Part model, mm, in its own coordinate system. A direction names the side the tool comes from. Round coordinates to 2 decimals unless told otherwise and drop trailing zeros. Loops run counter-clockwise (first coordinate to the right, second up) from the corner with the lowest first, then second, coordinate; pieces in that order, holes last.
from build123d import *

# Parameters (mm, degrees)
SKETCH_1_W                     = 248
SKETCH_1_H                     = 60
EXTRUDE_1_DEPTH                = 6
HOLE_WIZARD_M5_1_D             = 4.2
HOLE_WIZARD_M5_1_DEPTH         = 12.4
HOLE_WIZARD_M5_1_TIP           = 1.2618073
CHAMFER_1_SIZE                 = 2
HOLE_WIZARD_M5_1_2_D           = 5.5
HOLE_WIZARD_M5_1_2_DEPTH       = 12.4
HOLE_WIZARD_M5_1_2_CBORE_D     = 10
HOLE_WIZARD_M5_1_2_CBORE_DEPTH = 5.7
HOLE_WIZARD_M5_1_2_TIP         = 1.652366702


with BuildPart() as part:
    # 草图1 → 凸台-拉伸1 (new, symmetric)
    with BuildSketch(Plane.XY):
        Rectangle(SKETCH_1_W, SKETCH_1_H)
    extrude(amount=EXTRUDE_1_DEPTH, both=True)

    # Hole Wizard M5 _1
    with Locations(Plane.ZY.offset(124)):
        with Locations((0, 20), (0, -20)):
            Hole(HOLE_WIZARD_M5_1_D / 2, depth=HOLE_WIZARD_M5_1_DEPTH)
            with Locations((0, 0, -(HOLE_WIZARD_M5_1_DEPTH + HOLE_WIZARD_M5_1_TIP / 2))):  # 118° drill point
                Cone(0, HOLE_WIZARD_M5_1_D / 2, HOLE_WIZARD_M5_1_TIP, mode=Mode.SUBTRACT)

    # 倒角1
    chamfer_1_edges = [part.edges().sort_by_distance(p)[0] for p in [
        (124, -30, 0),
        (124, 30, 0),
    ]]
    chamfer(chamfer_1_edges, length=CHAMFER_1_SIZE)

    # Hole Wizard M5 _1 2
    with Locations(Plane(origin=(0, 0, -6), x_dir=(-1, 0, 0), z_dir=(0, 0, -1))):
        with Locations((-90, 0), (0, 0), (90, 0)):
            CounterBoreHole(HOLE_WIZARD_M5_1_2_D / 2, HOLE_WIZARD_M5_1_2_CBORE_D / 2, HOLE_WIZARD_M5_1_2_CBORE_DEPTH, depth=HOLE_WIZARD_M5_1_2_DEPTH)
            with Locations((0, 0, -(HOLE_WIZARD_M5_1_2_DEPTH + HOLE_WIZARD_M5_1_2_TIP / 2))):  # 118° drill point
                Cone(0, HOLE_WIZARD_M5_1_2_D / 2, HOLE_WIZARD_M5_1_2_TIP, mode=Mode.SUBTRACT)


solid = part.part
1) Mould opens along Y. For faces 1 (the face through (85.381, -1.915, -3.19)), 2 (the face through (-3, 30, 0)), 3 (the face through (-2, 7, -6)) say: released by +Y, released by -Y, zero draft, split by the parting line, or undercut.
Values:
face 1: undercut
face 2: released by +Y
face 3: zero draft
2) Slice it at A-A, the plane x = -90. Give the cut face in (y, z), then the cut area to 3 significant figures.
Values:
outline: (-30, -6) - (-5, -6) - (-5, -0.3) - (-2.75, -0.3) - (-2.75, 6) - (-30, 6) - close; (2.75, -0.3) - (5, -0.3) - (5, -6) - (30, -6) - (30, 6) - (2.75, 6) - close
area: 628 mm2
3) Wall check: line 1 along Y through (x, z) = (90, 2); line 2 along X through (y, z) = (-1, 5.5); line 3 along Y through (x, z) = (90, -3.05). Give the ranges that are in metal, low to high.
Values:
line 1: y = -30 to -2.75, 2.75 to 30
line 2: x = -124 to -92.56, -87.44 to -2.56, 2.56 to 87.44, 92.56 to 124
line 3: y = -30 to -5, 5 to 30
4) Drop flat-ended pins along their axis: pin 1 Ø5.5 at (y, z) = (-20, 0) entering from -X; pin 2 Ø9 at (x, y) = (0, 0) entering from -Z. Give the stop position or say it passes through.
Values:
pin 1: stops at x = -124
pin 2: stops at z = -0.3
5) Tool access for faces 4 (the face through (-117.71, -18.23, -1.13)), 5 (the face through (-92.2, -2.2, -0.3)), 6 (the face through (-124, 0, 0)): list every direction of +Z, -Z, +X, -X, +Y, -Y with a clear straight run to the whole face (end or side of a thin tool).
Values:
face 4: -X
face 5: -Z
face 6: +Z, -Z, -X, +Y, -Y
